Geometry check sheet. Reference: the model listing, model coordinates, mm. Face numbers are marked on the shaded views. A direction names the side the tool comes from. Coordinates: 2 decimals unless noted, no trailing zeros. Write each loop counter-clockwise with the first axis right and the second up, starting at its lowest first coordinate (ties: lowest second). Pieces come first, ordered by that corner, then holes. Notation, with made-up numbers: (64.5, 65) -> (123.5, 65) arc R18 cw to (123.5, 89) -> close; hole circle Ø11 at (67, 26). An arc over 180 degrees is marked (long way). Answer in a Markdown table with one row per item. Add a question column.
1. Cross-section at A-A on x = -19. Record the cut outline in (y, z), and give its area (3 significant figures).
2. Mould release check, pull along X, two halves, no side actions. Record for the marked faces 1, 2 and 3: pulls with the +X half, pulls with the -X half, needs draft (parallel to the pull), parting line crosses it, or undercut.
3. Depth check by flat-ended pin: P1, Ø1, axis at x = 23.5, y = 14, coming from the -Z side; P2, Ø22, axis at x = 55, y = 8, coming from the -Z side; P3, Ø6.5, axis at x = -19, z = 30, coming from the -Y side; P4, Ø4.5, axis at x = 54, z = 30, coming from the +Y side. Enter the tip coordinate at first touch or a pass-through.
4. Set-up check for the marked faces 4, 5, 6 and 7: record each of +Z, -Z, +X, -X, +Y, -Y from which the full face is reachable in a straight line by a thin tool's end or side.
5. Scan lines: L1, parallel to Y at x = 17.5, z = 35.5; L2, parallel to Y at x = 36, z = 35; L3, parallel to Z at x = -23.5, y = 10. Record each from-to range of solid material in increasing order. Write a range as from..to.
6. Cross-section at B-B on z = 22. Record the cut outline in (x, y), and give its area (3 significant figures).
7. Cross-section at C-C on y = 3. Record the cut outline in (x, z), and give its area (3 significant figures).
8. Cross-section at D-D on y = 25. Record the cut outline in (x, z).
```python
from build123d import *

# Parameters (mm, degrees)
BASE_BODY_DEPTH             = 40
MOUNTING_LUG_1_DEPTH        = 20
MOUNTING_LUG_2_DEPTH        = 20
LUG_2_BOTTOM_SLOT_PROFILE_W = 18
LUG_2_BOTTOM_SLOT_PROFILE_H = 6
LUG_2_BOTTOM_SLOT_DEPTH     = 20
LUG_1_BOTTOM_SLOT_PROFILE_W = 18
LUG_1_BOTTOM_SLOT_PROFILE_H = 6
LUG_1_BOTTOM_SLOT_DEPTH     = 20
LUG_2_HOLE_7_SKETCH_R       = 3.5
LUG_2_HOLE_7_DEPTH          = 7
LUG_2_HOLE_5_SKETCH_R       = 2.5
LUG_2_HOLE_5_DEPTH          = 7
LUG_1_HOLE_7_SKETCH_R       = 3.5
LUG_1_HOLE_7_DEPTH          = 7
LUG_1_HOLE_5_SKETCH_R       = 2.5
LUG_1_HOLE_5_DEPTH          = 7
BEARING_BORE_29_SKETCH_R    = 14.5
BEARING_BORE_29_DEPTH       = 30
THROUGH_BORE_21_SKETCH_R    = 10.5
THROUGH_BORE_21_DEPTH       = 87.02325267


with BuildPart() as part:
    # Base Body Profile → Base Body (new body)
    with BuildSketch(Plane.XY):
        Polygon((0, 0), (35, 0), (35, 35), (30, 40), (5, 40), (0, 35), align=None)
    extrude(amount=BASE_BODY_DEPTH)

    # Mounting Lug 1 Profile → Mounting Lug 1 (add)
    with BuildSketch(Plane.XY.offset(40)):
        Polygon((0, 0), (0, 20), (-19, 20), (-28, 20), (-30, 20), (-35, 15), (-35, 0), align=None)
    extrude(amount=-MOUNTING_LUG_1_DEPTH)

    # Mounting Lug 2 Profile → Mounting Lug 2 (add)
    with BuildSketch(Plane.XY.offset(40)):
        Polygon((35, 0), (35, 20), (54, 20), (63, 20), (65, 20), (70, 15), (70, 0), align=None)
    extrude(amount=-MOUNTING_LUG_2_DEPTH)

    # Lug 2 Bottom Slot Profile → Lug 2 Bottom Slot (cut)
    with BuildSketch(Plane(origin=(0, 0, 20), x_dir=(-1, 0, 0), z_dir=(0, 0, -1))):
        with Locations((-54, 3)):
            Rectangle(LUG_2_BOTTOM_SLOT_PROFILE_W, LUG_2_BOTTOM_SLOT_PROFILE_H)
    extrude(amount=-LUG_2_BOTTOM_SLOT_DEPTH, mode=Mode.SUBTRACT)

    # Lug 1 Bottom Slot Profile → Lug 1 Bottom Slot (cut)
    with BuildSketch(Plane(origin=(0, 0, 20), x_dir=(-1, 0, 0), z_dir=(0, 0, -1))):
        with Locations((19, 3)):
            Rectangle(LUG_1_BOTTOM_SLOT_PROFILE_W, LUG_1_BOTTOM_SLOT_PROFILE_H)
    extrude(amount=-LUG_1_BOTTOM_SLOT_DEPTH, mode=Mode.SUBTRACT)

    # Lug 2 Hole Ø7 Sketch → Lug 2 Hole Ø7 (cut)
    with BuildSketch(Plane(origin=(0, 20, 0), x_dir=(1, 0, 0), z_dir=(0, 1, 0))):
        with Locations(Location((54, -30, 0), (0, 0, 270))):
            Circle(LUG_2_HOLE_7_SKETCH_R)
    extrude(amount=-LUG_2_HOLE_7_DEPTH, mode=Mode.SUBTRACT)

    # Lug 2 Hole Ø5 Sketch → Lug 2 Hole Ø5 (cut)
    with BuildSketch(Plane(origin=(0, 13, 0), x_dir=(1, 0, 0), z_dir=(0, 1, 0))):
        with Locations(Location((54, -30, 0), (0, 0, 270))):
            Circle(LUG_2_HOLE_5_SKETCH_R)
    extrude(amount=-LUG_2_HOLE_5_DEPTH, mode=Mode.SUBTRACT)

    # Lug 1 Hole Ø7 Sketch → Lug 1 Hole Ø7 (cut)
    with BuildSketch(Plane(origin=(0, 20, 0), x_dir=(1, 0, 0), z_dir=(0, 1, 0))):
        with Locations(Location((-19, -30, 0), (0, 0, 270))):
            Circle(LUG_1_HOLE_7_SKETCH_R)
    extrude(amount=-LUG_1_HOLE_7_DEPTH, mode=Mode.SUBTRACT)

    # Lug 1 Hole Ø5 Sketch → Lug 1 Hole Ø5 (cut)
    with BuildSketch(Plane(origin=(0, 13, 0), x_dir=(1, 0, 0), z_dir=(0, 1, 0))):
        with Locations(Location((-19, -30, 0), (0, 0, 270))):
            Circle(LUG_1_HOLE_5_SKETCH_R)
    extrude(amount=-LUG_1_HOLE_5_DEPTH, mode=Mode.SUBTRACT)

    # Bearing Bore Ø29 Sketch → Bearing Bore Ø29 (cut)
    with BuildSketch(Plane(origin=(0, 0, 0), x_dir=(-1, 0, 0), z_dir=(0, 0, -1))):
        with Locations((-17.5, 25)):
            Circle(BEARING_BORE_29_SKETCH_R)
    extrude(amount=-BEARING_BORE_29_DEPTH, mode=Mode.SUBTRACT)

    # Through Bore Ø21 Sketch → Through Bore Ø21 (cut, through all)
    with BuildSketch(Plane(origin=(0, 0, 30), x_dir=(-1, 0, 0), z_dir=(0, 0, -1))):
        with Locations((-17.5, 25)):
            Circle(THROUGH_BORE_21_SKETCH_R)
    extrude(amount=-THROUGH_BORE_21_DEPTH, mode=Mode.SUBTRACT)


solid = part.part
```
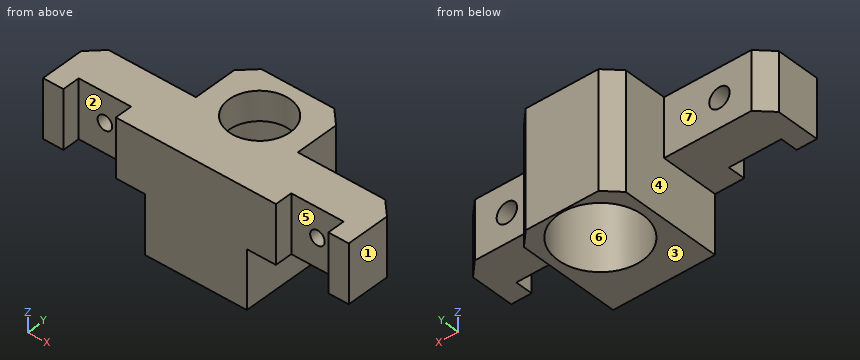
Results found:
| question | item | result |
|---|---|---|
| 1 | outline | (6, 20) -> (20, 20) -> (20, 26.5) -> (13, 26.5) -> (13, 27.5) -> (6, 27.5) -> close; (6, 32.5) -> (13, 32.5) -> (13, 33.5) -> (20, 33.5) -> (20, 40) -> (6, 40) -> close |
| 1 | area | 196 mm^2 |
| 2 | face 1 | pulls with the +X half |
| 2 | face 2 | undercut |
| 2 | face 3 | needs draft |
| 3 | P1 | stops at z = 30 |
| 3 | P2 | stops at z = 20 |
| 3 | P3 | stops at y = 6 |
| 3 | P4 | passes through |
| 4 | face 4 | -Z, -X, +Y |
| 4 | face 5 | +Z, -Z, -Y |
| 4 | face 6 | -Z |
| 4 | face 7 | +Z, -Z, -X, +Y |
| 5 | L1 | y = 0..14.5, 35.5..40 |
| 5 | L2 | y = 0..20 |
| 5 | L3 | z = 20..40 |
| 6 | outline | (-35, 0) -> (-28, 0) -> (-28, 6) -> (-10, 6) -> (-10, 0) -> (45, 0) -> (45, 6) -> (63, 6) -> (63, 0) -> (70, 0) -> (70, 15) -> (65, 20) -> (35, 20) -> (35, 35) -> (30, 40) -> (5, 40) -> (0, 35) -> (0, 20) -> (-30, 20) -> (-35, 15) -> close; hole circle Ø29 at (17.5, 25) |
| 6 | area | 1,870 mm^2 |
| 7 | outline | (-35, 20) -> (-28, 20) -> (-28, 40) -> (-35, 40) -> close; (-10, 20) -> (0, 20) -> (0, 0) -> (35, 0) -> (35, 20) -> (45, 20) -> (45, 40) -> (-10, 40) -> close; (63, 20) -> (70, 20) -> (70, 40) -> (63, 40) -> close |
| 7 | area | 2,080 mm^2 |
| 8 | outline | (0, 0) -> (3, 0) -> (3, 30) -> (7, 30) -> (7, 40) -> (0, 40) -> close; (28, 30) -> (32, 30) -> (32, 0) -> (35, 0) -> (35, 40) -> (28, 40) -> close |
